```python
from build123d import *

# Parameters (mm, degrees)
SKETCH1_W           = 20
SKETCH1_H           = 20
SKETCH1_R           = 1.5
SKETCH1_R_2         = 3
BOSS_EXTRUDE1_DEPTH = 10
CUT_EXTRUDE5_START  = 10
SKETCH1_3_R         = 1.5
CUT_EXTRUDE5_DEPTH  = 5
SKETCH2_R           = 3
CUT_EXTRUDE1_DEPTH  = 31
SKETCH3_R           = 1.5
CUT_EXTRUDE2_DEPTH  = 3.5
FILLET1_R           = 0.1


with BuildPart() as part:
    # Sketch1 → Boss-Extrude1 (new body)
    # profile 1 of 2: a face of its own
    with BuildSketch(Plane(origin=(0, 0, 0), x_dir=(1, 0, 0), z_dir=(0, 1, 0))):
        with Locations((10, 10)):
            Rectangle(SKETCH1_W, SKETCH1_H)
        with Locations((6, 10)):
            Circle(SKETCH1_R, mode=Mode.SUBTRACT)
        with Locations(Location((14, 10, 0), (0, 0, 270))):
            Circle(SKETCH1_R_2, mode=Mode.SUBTRACT)
    # profile 2 of 2: a face of its own
    with BuildSketch(Plane(origin=(0, 0, 0), x_dir=(1, 0, 0), z_dir=(0, 1, 0))):
        with Locations((6, 10)):
            Circle(SKETCH1_R)
    extrude(amount=BOSS_EXTRUDE1_DEPTH)

    # Sketch1<3> → Cut-Extrude5 (cut)
    with BuildSketch(Plane(origin=(0, 0, 0), x_dir=(1, 0, 0), z_dir=(0, 1, 0)).offset(CUT_EXTRUDE5_START)):
        with Locations(Location((6, 10, 0), (0, 0, 270))):
            Circle(SKETCH1_3_R)
    extrude(amount=-CUT_EXTRUDE5_DEPTH, mode=Mode.SUBTRACT)

    # Sketch2 → Cut-Extrude1 (cut, through all)
    with BuildSketch(Plane.XY):
        with Locations((6, 5)):
            Circle(SKETCH2_R)
    extrude(amount=-CUT_EXTRUDE1_DEPTH, mode=Mode.SUBTRACT)

    # Sketch3 → Cut-Extrude2 (cut)
    with BuildSketch(Plane.XY):
        with Locations((14, 5)):
            Circle(SKETCH3_R)
    extrude(amount=-CUT_EXTRUDE2_DEPTH, mode=Mode.SUBTRACT)

    # Fillet1
    fillet1_edges = [part.edges().sort_by_distance(p)[0] for p in [
        (20, 10, -10),
        (10, 10, -20),
        (0, 10, -10),
        (0, 0, -10),
        (10, 0, -20),
        (20, 0, -10),
        (10, 0, 0),
        (10, 10, 0),
    ]]
    fillet(fillet1_edges, radius=FILLET1_R)


solid = part.part
```
The listing builds one solid part. Answer for the finished solid, in the listing's coordinates (mm). A direction names the side the tool comes from. Coordinates: 2 decimals unless noted, no trailing zeros. Write each loop counter-clockwise with the first axis right and the second up, starting at its lowest first coordinate (ties: lowest second). Pieces come first, ordered by that corner, then holes. Notation, with made-up numbers: (7, 24.5) - (41, 24.5) arc R14 cw to (41, 28.5) - close; hole circle Ø1 at (10.5, 81). An arc over 180 degrees is marked (long way). Return JSON: item names as keys, results as strings. Group by question number.
1. Given pin 1 (0.9 mm diameter, centred on x = 13.5, y = 5.5, fed in from +Z); pin 2 (5 mm diameter, centred on x = 14, z = -10, fed in from -Y), each flat-ended and moving along its own axis, determine where each tip first touches the part or whether it passes through.
2. Straight lines are drawn through the part: L1, parallel to X at y = 9.05, z = -10; L2, parallel to X at y = 6, z = -11; L3, parallel to Z at x = 6, y = 9.3. For each, find the intervals that lie inside material, in ascending order.
3. A cutting plane is placed at A-A, the plane y = 4.5. Determine the outline of the cut face in (x, z), plus the area to 3 significant figures.
4. A cutting plane is placed at D-D, the plane x = 6. Determine the outline of the cut face in (y, z).
5. Determine the mould class of faces 4 (the flat face through (10, 5, -20)), 5 (the flat face through (14, 5, -3.5)), 6 (the flat face through (0, 5, -10)), 7 (the flat face through (20, 5, -10)) for opening direction X: released by +X, released by -X, zero draft, split by the parting line, or undercut.
6. A cutting plane is placed at C-C, the plane z = -13.5. Determine the outline of the cut face in (x, y).
7. Which of the six approach directions +Z, -Z, +X, -X, +Y, -Y give full straight-line access (tool end or side, diameter ignored) to faces 1 (the cylindrical face through (5.35, 2.07, -9.86)), 2 (the cylindrical face through (5.425, 8.816, -8.614)), 3 (the cylindrical face through (12.5, 5.07, -1.73))?
8. A cutting plane is placed at B-B, the plane x = 14. Determine the outline of the cut face in (y, z).
Ans:
{
 "1": {"pin 1": "z = -3.5", "pin 2": "through"},
 "2": {"L1": "0 to 4.5, 7.5 to 11, 17 to 20", "L2": "0 to 3.17, 8.83 to 11.17, 16.83 to 20", "L3": "-20 to -11.5, -8.5 to 0"},
 "3": {"outline": "(0, -20) - (3.04, -20) - (3.04, 0) - (0, 0) - close; (8.96, -20) - (20, -20) - (20, 0) - (15.41, 0) - (15.41, -3.5) - (12.59, -3.5) - (12.59, 0) - (8.96, 0) - close; hole circle Ø6 at (14, -10)", "area": "244 mm²"},
 "4": {"outline": "(0, -19.9) arc R0.1 ccw to (0.1, -20) - (2, -20) - (2, 0) - (0.1, 0) arc R0.1 ccw to (0, -0.1) - close; (8, -20) - (9.9, -20) arc R0.1 ccw to (10, -19.9) - (10, -11.5) - (8, -11.5) - close; (8, -8.5) - (10, -8.5) - (10, -0.1) arc R0.1 ccw to (9.9, 0) - (8, 0) - close"},
 "5": {"face 4": "zero draft", "face 5": "undercut", "face 6": "released by -X", "face 7": "released by +X"},
 "6": {"outline": "(0, 0.1) arc R0.1 ccw to (0.1, 0) - (19.9, 0) arc R0.1 ccw to (20, 0.1) - (20, 9.9) arc R0.1 ccw to (19.9, 10) - (0.1, 10) arc R0.1 ccw to (0, 9.9) - close; hole circle Ø6 at (6, 5)"},
 "7": {"face 1": "+Z, -Z", "face 2": "+Y", "face 3": "+Z"},
 "8": {"outline": "(0, -19.9) arc R0.1 ccw to (0.1, -20) - (9.9, -20) arc R0.1 ccw to (10, -19.9) - (10, -13) - (0, -13) - close; (0, -7) - (10, -7) - (10, -0.1) arc R0.1 ccw to (9.9, 0) - (6.5, 0) - (6.5, -3.5) - (3.5, -3.5) - (3.5, 0) - (0.1, 0) arc R0.1 ccw to (0, -0.1) - close"}
}
